```python
from build123d import *

# Parameters (mm, degrees)
CHAMFER1_SIZE = 0.5


with BuildPart() as part:
    # Sketch1 → Revolve1 (revolve)
    with BuildSketch(Plane(origin=(0, 0, 0), x_dir=(0, 0, -1), z_dir=(1, 0, 0))):
        Polygon((0, 30), (3.05, 30), (3.05, 8), (5, 8), (5, 3), (7.5, 3), (7.5, 0), (0, 0), align=None)
    revolve(axis=Axis((0, 0, 0), (0, 1, 0)))

    # Chamfer1
    chamfer1_edges = [part.edges().sort_by_distance(p)[0] for p in [
        (0, 0, 7.5),
        (0, 3, 7.5),
        (0, 8, 5),
        (0, 30, 3.05),
    ]]
    chamfer(chamfer1_edges, length=CHAMFER1_SIZE)


solid = part.part
```
Here's how the part is built. I have some questions about the finished solid (model axes, mm). A direction names the side the tool comes from. Round coordinates to 2 decimals unless told otherwise and drop trailing zeros. Order: outer loops, then holes, each group sorted by start corner. A loop starts at its lowest first (then second) coordinate and runs counter-clockwise, first axis right, second up. Notation, with made-up numbers: (38, -22) -> (65, -22) arc R20 ccw to (65, 1) -> close; hole circle Ø2 at (64.5, 55). An arc over 180 degrees is marked (long way). Use a Markdown table: item, result. Add a question column.
(1) Suppose I cut it at B-B, the plane x = 0. Please give me the cut outline in (y, z).
(2) Suppose I cut it at A-A, the plane z = 0. Please give me the cut outline in (x, y), and give its area (3 significant figures).
(3) Suppose I cut it at C-C, the plane y = 16.75. Please give me the cut outline in (x, z).
(4) For faces 1 (the face through (0, 30, 0)), 2 (the face through (-0.134, 18.6, 3.047)), which set-ups out of +Z, -Z, +X, -X, +Y, -Y let a thin tool reach every point of the face, with its end or its side?
(5) Suppose I cut it at D-D, the plane y = 7. Please give me the cut outline in (x, z), and give its area (3 significant figures).
(6) For pin 1 Ø4 at (y, z) = (12, 0) entering from +X; pin 2 Ø4 at (x, y) = (3, 27) entering from +Z; pin 3 Ø1.5 at (y, z) = (16, 2.5) entering from +X, each with a flat end and sliding along its axis, tell me the tip position at first contact or that it passes through.
(7) I need wall thicknesses on line 1 along Y through (x, z) = (4.75, 1.75); line 2 along Z through (x, y) = (0, 14.25). Which ranges of each line are inside material? Lowest first, please.
Verdict:
| question | item | result |
|---|---|---|
| 1 | outline | (0, -7) -> (0.5, -7.5) -> (2.5, -7.5) -> (3, -7) -> (3, -5) -> (7.5, -5) -> (8, -4.5) -> (8, -3.05) -> (29.5, -3.05) -> (30, -2.55) -> (30, 2.55) -> (29.5, 3.05) -> (8, 3.05) -> (8, 4.5) -> (7.5, 5) -> (3, 5) -> (3, 7) -> (2.5, 7.5) -> (0.5, 7.5) -> (0, 7) -> close |
| 2 | outline | (-7.5, 0.5) -> (-7, 0) -> (7, 0) -> (7.5, 0.5) -> (7.5, 2.5) -> (7, 3) -> (5, 3) -> (5, 7.5) -> (4.5, 8) -> (3.05, 8) -> (3.05, 29.5) -> (2.55, 30) -> (-2.55, 30) -> (-3.05, 29.5) -> (-3.05, 8) -> (-4.5, 8) -> (-5, 7.5) -> (-5, 3) -> (-7, 3) -> (-7.5, 2.5) -> close |
| 2 | area | 228 mm2 |
| 3 | outline | circle Ø6.1 at (0, 0) |
| 4 | face 1 | +Z, -Z, +X, -X, +Y |
| 4 | face 2 | +Y |
| 5 | outline | circle Ø10 at (0, 0) |
| 5 | area | 78.5 mm2 |
| 6 | pin 1 | x = 3.05 |
| 6 | pin 2 | z = 2.88 |
| 6 | pin 3 | x = 2.5 |
| 7 | line 1 | 0 to 3 |
| 7 | line 2 | -3.05 to 3.05 |
